Verification items for this drawing (mm, ordinates from the low corner). A direction names the side the tool comes from. Round coordinates to 2 decimals unless told otherwise and drop trailing zeros. Order: outer loops, then holes, each group sorted by start corner. A loop starts at its lowest first (then second) coordinate and runs counter-clockwise, first axis right, second up. Notation, with made-up numbers: (-32, -30.5) -> (12, -30.5) arc R31 cw to (12, -6.5) -> close; hole circle Ø4 at (-4.5, 82.25). An arc over 180 degrees is marked (long way). Answer in a Markdown table with one row per item. Add a question column.
1. Sectioned sample at C-C, the plane x = 15. Record the boundary of the cut face in (y, z).
2. Material ranges on L1, parallel to Z at x = 165, y = 11; L2, parallel to X at y = 7, z = 15; L3, parallel to X at y = 10, z = 40, recorded low to high. Write a range as from..to.
3. Depth check by flat-ended pin: P1, Ø3, axis at x = 134, y = 37, coming from the +Z side; P2, Ø3, axis at y = 26, z = 20.5, coming from the +X side; P3, Ø25, axis at x = 126, y = 27.5, coming from the +Z side; P4, Ø15, axis at x = 165.5, z = 34.5, coming from the +Y side. Enter the tip coordinate at first touch or a pass-through.
4. Sectioned sample at D-D, the plane x = 90. Record the boundary of the cut face in (y, z).
5. Access from +Z, -Z, +X, -X, +Y, -Y to the whole of each face (thin tool, end or side, straight path). Record for the marked faces 1, 2 and 3.
6. Sectioned sample at A-A, the plane z = 40.5. Record the boundary of the cut face in (x, y), then the cut area to 3 significant figures.
7. Sectioned sample at B-B, the plane y = 5. Record the boundary of the cut face in (x, z), then the cut area to 3 significant figures.
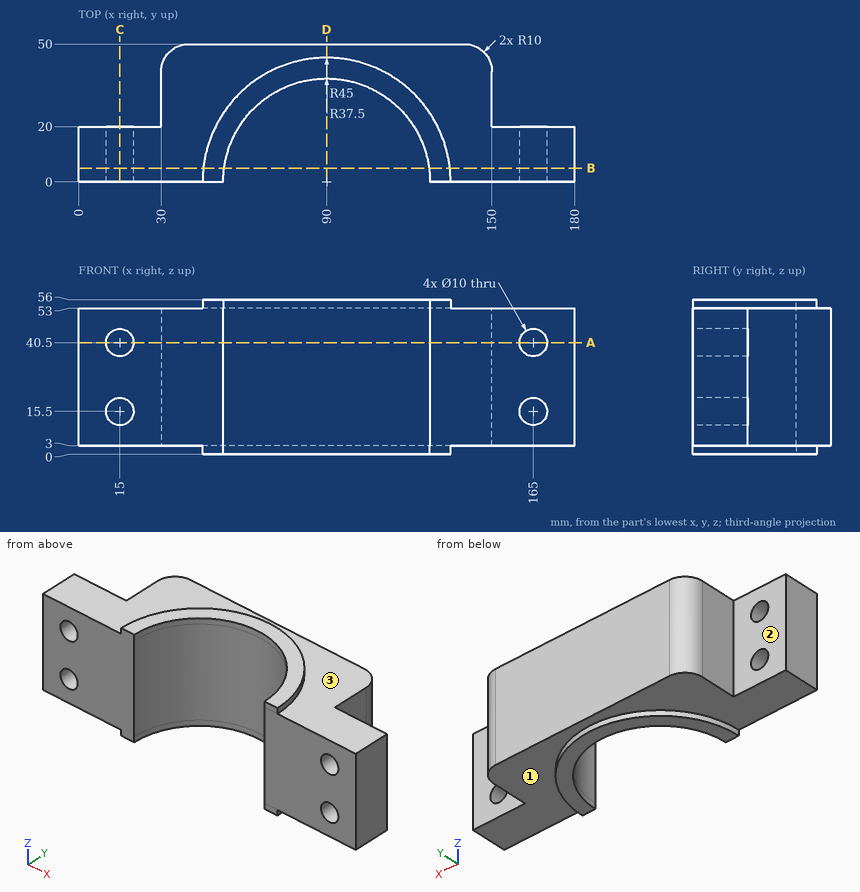
Answer key:
| question | item | result |
|---|---|---|
| 1 | outline | (0, 3) -> (20, 3) -> (20, 10.5) -> (0, 10.5) -> close; (0, 20.5) -> (20, 20.5) -> (20, 35.5) -> (0, 35.5) -> close; (0, 45.5) -> (20, 45.5) -> (20, 53) -> (0, 53) -> close |
| 2 | L1 | z = 3..10.5, 20.5..35.5, 45.5..53 |
| 2 | L2 | x = 0..10.03, 19.97..53.16, 126.84..160.03, 169.97..180 |
| 2 | L3 | x = 0..10.03, 19.97..53.86, 126.14..160.03, 169.97..180 |
| 3 | P1 | stops at z = 53 |
| 3 | P2 | stops at x = 150 |
| 3 | P3 | stops at z = 56 |
| 3 | P4 | stops at y = 20 |
| 4 | outline | (37.5, 0) -> (45, 0) -> (45, 3) -> (50, 3) -> (50, 53) -> (45, 53) -> (45, 56) -> (37.5, 56) -> close |
| 5 | face 1 | -Z, +Y |
| 5 | face 2 | +Z, -Z, -X, +Y |
| 5 | face 3 | +Z, +Y |
| 6 | outline | (0, 0) -> (10, 0) -> (10, 20) -> (0, 20) -> close; (20, 0) -> (52.5, 0) arc R37.5 cw to (127.5, 0) -> (160, 0) -> (160, 20) -> (150, 20) -> (150, 40) arc R10 ccw to (140, 50) -> (40, 50) arc R10 ccw to (30, 40) -> (30, 20) -> (20, 20) -> close; (170, 0) -> (180, 0) -> (180, 20) -> (170, 20) -> close |
| 6 | area | 4,550 mm² |
| 7 | outline | (0, 3) -> (45.28, 3) -> (45.28, 0) -> (52.83, 0) -> (52.83, 56) -> (45.28, 56) -> (45.28, 53) -> (0, 53) -> close; (127.17, 0) -> (134.72, 0) -> (134.72, 3) -> (180, 3) -> (180, 53) -> (134.72, 53) -> (134.72, 56) -> (127.17, 56) -> close; hole circle Ø10 at (15, 15.5); hole circle Ø10 at (15, 40.5); hole circle Ø10 at (165, 15.5); hole circle Ø10 at (165, 40.5) |
| 7 | area | 5,060 mm² |
